Source: CAD feature listing. Evaluate the final solid. Frame: model axes, mm. A direction names the side the tool comes from. Give positions to 0.01 mm unless a question says otherwise; leave off trailing zeros. Order: outer loops, then holes, each group sorted by start corner. A loop starts at its lowest first (then second) coordinate and runs counter-clockwise, first axis right, second up.
from build123d import *
from build123d.topology import SkipClean

# Parameters (mm, degrees)
BOSS_EXTRUDE1_DEPTH          = 5
SKETCH2_R                    = 2.5
BOSS_EXTRUDE2_DEPTH          = 7
SKETCH4_R                    = 2.5
BOSS_EXTRUDE4_DEPTH          = 9
SKETCH10_R                   = 2.5
BOSS_EXTRUDE6_DEPTH          = 5
SKETCH13_W                   = 0.75
SKETCH13_H                   = 0.75
CUT_REVOLVE1_ANGLE           = 45
CUT_REVOLVE1_OTHER_WAY_ANGLE = 45
SKETCH15_W                   = 0.75
SKETCH15_H                   = 0.75
CUT_REVOLVE2_ANGLE           = 45
CUT_REVOLVE2_OTHER_WAY_ANGLE = 45
SKETCH17_R                   = 4
BOSS_EXTRUDE7_DEPTH          = 5
SKETCH18_R                   = 2.930859256
CUT_EXTRUDE1_DEPTH           = 7
SKETCH19_R                   = 2.625
CUT_EXTRUDE2_DEPTH           = 7
SKETCH20_R                   = 4
BOSS_EXTRUDE8_DEPTH          = 5
SKETCH21_R                   = 2.625
CUT_EXTRUDE3_DEPTH           = 50.162013496
SKETCH23_R                   = 4
BOSS_EXTRUDE9_DEPTH          = 5
SKETCH24_R                   = 2.625
CUT_EXTRUDE4_DEPTH           = 15
CUT_EXTRUDE5_DEPTH           = 10
CUT_EXTRUDE6_DEPTH           = 48.390965078
BOSS_EXTRUDE10_DEPTH         = 5


with BuildPart() as part:
    # Sketch1 → Boss-Extrude1 (new body)
    with BuildSketch(Plane.XY):
        with BuildLine():
            Line((1, 0), (44, 0))
            ThreePointArc((44, 0), (44.707106781, -0.292893219), (45, -1))
            Line((45, -1), (45, -4))
            ThreePointArc((45, -4), (44.707106781, -4.707106781), (44, -5))
            Line((44, -5), (1, -5))
            ThreePointArc((1, -5), (0.292893219, -4.707106781), (0, -4))
            Line((0, -4), (0, -1))
            ThreePointArc((0, -1), (0.292893219, -0.292893219), (1, 0))
        make_face()
    extrude(amount=BOSS_EXTRUDE1_DEPTH)

    # Sketch2 → Boss-Extrude2 (add)
    with BuildSketch(Plane(origin=(0, 0, 0), x_dir=(-1, 0, 0), z_dir=(0, 0, -1))):
        with Locations(Location((-42.676049222, -2.5, 0), (0, 0, 158.369487395))):
            Circle(SKETCH2_R)
    extrude(amount=BOSS_EXTRUDE2_DEPTH)

    # Sketch4 → Boss-Extrude4 (add)
    with BuildSketch(Plane.XY.offset(5)):
        with Locations(Location((35, -2.5, 0), (0, 0, 270))):
            Circle(SKETCH4_R)
    extrude(amount=BOSS_EXTRUDE4_DEPTH)

    # Sketch10 → Boss-Extrude6 (add)
    with BuildSketch(Plane.XY.offset(5)):
        with Locations(Location((4.676049222, -2.5, 0), (0, 0, 270))):
            Circle(SKETCH10_R)
    extrude(amount=BOSS_EXTRUDE6_DEPTH)

    # Sketch13 → Cut-Revolve1 (revolve, cut)
    with BuildSketch(Plane(origin=(35, 0, 1.995810748), x_dir=(0, 1, 0), z_dir=(1, 0, 0))):
        with Locations((-0.375, 8.375)):
            Rectangle(SKETCH13_W, SKETCH13_H)
        with Locations((-4.625, 8.375)):
            Rectangle(SKETCH13_W, SKETCH13_H)
    revolve(axis=Axis((35, -2.5, 15.995810748), (0, 0, -1)), revolution_arc=CUT_REVOLVE1_ANGLE, mode=Mode.SUBTRACT)

    # Sketch13 → Cut-Revolve1 other way (revolve, cut)
    with BuildSketch(Plane(origin=(35, 0, 1.995810748), x_dir=(0, 1, 0), z_dir=(1, 0, 0))):
        with Locations((-0.375, 8.375)):
            Rectangle(SKETCH13_W, SKETCH13_H)
        with Locations((-4.625, 8.375)):
            Rectangle(SKETCH13_W, SKETCH13_H)
    revolve(axis=Axis((35, -2.5, 15.995810748), (0, 0, 1)), revolution_arc=CUT_REVOLVE1_OTHER_WAY_ANGLE, mode=Mode.SUBTRACT)

    # Sketch15 → Cut-Revolve2 (revolve, cut)
    with BuildSketch(Plane(origin=(42.676049222, 0, -1.99986967), x_dir=(0, 1, 0), z_dir=(-1, 0, 0))):
        with Locations((-0.375, 3.375)):
            Rectangle(SKETCH15_W, SKETCH15_H)
        with Locations((-4.625, 3.375)):
            Rectangle(SKETCH15_W, SKETCH15_H)
    revolve(axis=Axis((42.676049222, -2.5, -8.99986967), (0, 0, 1)), revolution_arc=CUT_REVOLVE2_ANGLE, mode=Mode.SUBTRACT)

    # Sketch15 → Cut-Revolve2 other way (revolve, cut)
    with BuildSketch(Plane(origin=(42.676049222, 0, -1.99986967), x_dir=(0, 1, 0), z_dir=(-1, 0, 0))):
        with Locations((-0.375, 3.375)):
            Rectangle(SKETCH15_W, SKETCH15_H)
        with Locations((-4.625, 3.375)):
            Rectangle(SKETCH15_W, SKETCH15_H)
    revolve(axis=Axis((42.676049222, -2.5, -8.99986967), (0, 0, -1)), revolution_arc=CUT_REVOLVE2_OTHER_WAY_ANGLE, mode=Mode.SUBTRACT)

    # Sketch17 → Boss-Extrude7 (add)
    with BuildSketch(Plane.XY.offset(5)):
        with Locations((42.676049222, -2.5)):
            Circle(SKETCH17_R)
    extrude(amount=-BOSS_EXTRUDE7_DEPTH)

    # Sketch18 → Cut-Extrude1 (cut)
    with BuildSketch(Plane(origin=(0, 0, -7), x_dir=(-1, 0, 0), z_dir=(0, 0, -1))):
        with Locations((-42.676049222, -2.5)):
            Circle(SKETCH18_R)
    extrude(amount=-CUT_EXTRUDE1_DEPTH, mode=Mode.SUBTRACT)

    # Sketch19 → Cut-Extrude2 (cut)
    with BuildSketch(Plane.XY.offset(5)):
        with Locations((42.676049222, -2.5)):
            Circle(SKETCH19_R)
    extrude(amount=-CUT_EXTRUDE2_DEPTH, mode=Mode.SUBTRACT)

    # Sketch20 → Boss-Extrude8 (add)
    with BuildSketch(Plane(origin=(0, 0, 0), x_dir=(-1, 0, 0), z_dir=(0, 0, -1))):
        with Locations((-35, -2.5)):
            Circle(SKETCH20_R)
    extrude(amount=-BOSS_EXTRUDE8_DEPTH)

    # Sketch21 → Cut-Extrude3 (cut, through all)
    with BuildSketch(Plane(origin=(0, 0, 0), x_dir=(-1, 0, 0), z_dir=(0, 0, -1))):
        with Locations((-35, -2.5)):
            Circle(SKETCH21_R)
    extrude(amount=-CUT_EXTRUDE3_DEPTH, mode=Mode.SUBTRACT)

    # Sketch23 → Boss-Extrude9 (add)
    with BuildSketch(Plane.XY.offset(5)):
        with Locations((4.676049222, -2.5)):
            Circle(SKETCH23_R)
    extrude(amount=-BOSS_EXTRUDE9_DEPTH)

    # Sketch24 → Cut-Extrude4 (cut)
    with BuildSketch(Plane.XY.offset(10)):
        with Locations((4.676049222, -2.5)):
            Circle(SKETCH24_R)
    extrude(amount=-CUT_EXTRUDE4_DEPTH, mode=Mode.SUBTRACT)

    # Sketch25 → Cut-Extrude5 (cut)
    with BuildSketch(Plane.XY.offset(5)):
        with BuildLine():
            Line((1.553550223, -5), (-1.854692679, -7.728778219))
            Line((-1.854692679, -7.728778219), (-3.436521983, -2.874938814))
            Line((-3.436521983, -2.874938814), (-1.53654244, 1.593813071))
            Line((-1.53654244, 1.593813071), (0.676049222, 3.037797523))
            Line((0.676049222, 3.037797523), (1.553550223, 0))
            ThreePointArc((1.553550223, 0), (0.676049222, -2.5), (1.553550223, -5))
        make_face()
    extrude(amount=-CUT_EXTRUDE5_DEPTH, mode=Mode.SUBTRACT)

    # Sketch26 → Cut-Extrude6 (cut, through all)
    with SkipClean():  # the faces are left unmerged after this step: merging them gives an invalid solid
        with BuildSketch(Plane.XY.offset(5)):
            Polygon((31, 2.88382286), (31, 2.910088177), (31.877501001, 0), (7.798548222, 0), align=None)
            with BuildLine():
                Line((39.403739803, 2.542373737), (38.122498999, 0))
                Line((38.122498999, 0), (39.553550223, 0))
                ThreePointArc((39.553550223, 0), (39.704808809, 0.178008664), (39.866200483, 0.346884273))
                Line((39.866200483, 0.346884273), (39.403739803, 2.542373737))
            make_face()
            with BuildLine():
                ThreePointArc((31.877501001, 0), (31.225745372, -1.175235115), (31, -2.5))
                Line((31, -2.5), (8.676049222, -2.5))
                ThreePointArc((8.676049222, -2.5), (8.450303851, -1.175235115), (7.798548222, 0))
                Line((7.798548222, 0), (31.877501001, 0))
            make_face()
            with BuildLine():
                Line((39.553550223, 0), (38.122498999, 0))
                ThreePointArc((38.122498999, 0), (38.547347694, -0.651669851), (38.838024611, -1.373249325))
                ThreePointArc((38.838024611, -1.373249325), (39.128701529, -0.651669851), (39.553550223, 0))
            make_face()
        extrude(amount=-CUT_EXTRUDE6_DEPTH, mode=Mode.SUBTRACT)

    # Sketch27 → Boss-Extrude10 (add, through all)
    with SkipClean():  # the faces are left unmerged after this step: merging them gives an invalid solid
        with BuildSketch(Plane.XY.offset(5)):
            Polygon((4.676049222, -6.5), (35, -6.5), (42.676049222, -6.5), (39.429079082, -3.966331103), (35, -5.966502381), (31.287082695, -3.966331103), (8.288836977, -3.966331103), align=None)
        extrude(amount=-BOSS_EXTRUDE10_DEPTH)


solid = part.part
(1) Section C-C, the plane x = 18. Return loops of the section in (y, z), plus the area to 3 significant figures.
(2) Pin query (flat end, axial travel): pin 1 Ø1.5 at (x, z) = (22.5, 1.5) entering from +Y; pin 2 Ø2 at (x, z) = (33, 4.5) entering from +Y; pin 3 Ø4 at (x, y) = (42.68, -2.5) entering from +Z. Return the tip coordinate at first contact, or that it passes through.
(3) Line query: line 1 along X through (y, z) = (-3.75, 4.45); line 2 along Y through (x, z) = (16, 3); line 3 along Y through (x, z) = (35.5, 3.1). Output: solid intervals per line, ascending.
(4) Section A-A, the plane x = 35. Return loops of the section in (y, z) (3 decimals).
(5) Draft query along X for faces 1 (the flat face through (23, -4, 0)), 2 (the cylindrical face through (45.18, -1.71, 2.54)). Return one class per face: +X half, -X half, draft (parallel to the pull), parting line (faces both ways), or undercut.
(6) Section B-B, the plane z = 3.5. Count the separate pieces of the cut face and the enclosed holes in it, plus the area to 3 significant figures.
(7) Access query for faces 3 (the flat face through (23, -6.5, 3)), 4 (the flat face through (20, -2.5, 3)). Directions: +Z, -Z, +X, -X, +Y, -Y. A direction counts if a zero-diameter tool reaches every point of the face in a straight line with its end or side. Return the directions, or none.
Checks:
1. outline: (-6.5, 0) - (-2.5, 0) - (-2.5, 5) - (-6.5, 5) - close
1. area: 20.0 mm2
2. pin 1: stops at y = -2.5
2. pin 2: stops at y = 1.37
2. pin 3: passes through
3. line 1: x = 0.88 to 2.37, 6.98 to 32.69, 37.31 to 40.37, 44.98 to 46.48
3. line 2: y = -6.5 to -2.5
3. line 3: y = -6.5 to -5.08, 0.08 to 1.47
4. outline: (-6.5, 0) - (-5.125, 0) - (-5.125, 5) - (-6.5, 5) - close; (0.125, 0) - (1.5, 0) - (1.5, 5) - (0.125, 5) - close
5. face 1: draft
5. face 2: undercut
6. separate pieces: 1
6. enclosed holes: 3
6. area: 187 mm2
7. face 3: +Z, -Z, +X, -X, -Y
7. face 4: +Z, -Z, +Y
